```python
from build123d import *

# Parameters (mm, degrees)
SKETCH_1_W                    = 140
SKETCH_1_H                    = 140
EXTRUDE_1_DEPTH               = 24
SKETCH_2_R                    = 27.5
CUT_EXTRUDE_1_DEPTH           = 22
SKETCH_3_R                    = 24.5
CUT_EXTRUDE_2_DEPTH           = 102.410058673
HOLE_WIZARD_M10_1_D           = 12
HOLE_WIZARD_M10_1_CBORE_D     = 18
HOLE_WIZARD_M10_1_CBORE_DEPTH = 10.6
CHAMFER_1_SIZE                = 10
HOLE_WIZARD_M6_1_D            = 5
SKETCH_11_R                   = 40
CUT_EXTRUDE_3_DEPTH           = 9


with BuildPart() as part:
    # 草图1 → 凸台-拉伸1 (new body)
    with BuildSketch(Plane.XY):
        Rectangle(SKETCH_1_W, SKETCH_1_H)
    extrude(amount=EXTRUDE_1_DEPTH)

    # 草图2 → 切除-拉伸1 (cut)
    with BuildSketch(Plane(origin=(0, 0, 0), x_dir=(-1, 0, 0), z_dir=(0, 0, -1))):
        Circle(SKETCH_2_R)
    extrude(amount=-CUT_EXTRUDE_1_DEPTH, mode=Mode.SUBTRACT)

    # 草图3 → 切除-拉伸2 (cut, through all)
    with BuildSketch(Plane(origin=(0, 0, 22), x_dir=(-1, 0, 0), z_dir=(0, 0, -1))):
        Circle(SKETCH_3_R)
    extrude(amount=-CUT_EXTRUDE_2_DEPTH, mode=Mode.SUBTRACT)

    # M10 六角凹头螺钉的柱形沉头孔1 (through all)
    with Locations(Plane(origin=(0, 0, 0), x_dir=(-1, 0, 0), z_dir=(0, 0, -1))):
        with Locations((-52.5, 52.5), (52.5, 52.5), (52.5, -52.5), (-52.5, -52.5)):
            CounterBoreHole(HOLE_WIZARD_M10_1_D / 2, HOLE_WIZARD_M10_1_CBORE_D / 2, HOLE_WIZARD_M10_1_CBORE_DEPTH)

    # 倒角1
    chamfer_1_edges = [part.edges().sort_by_distance(p)[0] for p in [
        (70, -70, 12),
        (-70, -70, 12),
        (-70, 70, 12),
        (70, 70, 12),
    ]]
    chamfer(chamfer_1_edges, length=CHAMFER_1_SIZE)

    # M6 螺纹孔1 (through all)
    with Locations(Plane(origin=(0, 0, 0), x_dir=(-1, 0, 0), z_dir=(0, 0, -1))):
        with Locations((-35, 35), (35, 35), (35, -35), (-35, -35), (0, 0)):
            Hole(HOLE_WIZARD_M6_1_D / 2)

    # 草图11 → 切除-拉伸3 (cut)
    with BuildSketch(Plane(origin=(0, 0, 0), x_dir=(-1, 0, 0), z_dir=(0, 0, -1))):
        Circle(SKETCH_11_R)
    extrude(amount=-CUT_EXTRUDE_3_DEPTH, mode=Mode.SUBTRACT)


solid = part.part
```
Read the model definition and answer for the solid it produces. Units are mm, in the model's axes. A direction names the side the tool comes from. Give positions to 0.01 mm unless a question says otherwise; leave off trailing zeros. Order: outer loops, then holes, each group sorted by start corner. A loop starts at its lowest first (then second) coordinate and runs counter-clockwise, first axis right, second up.
(1) For a pull along X with two mould halves and no side action, classify faces 3 (the cylindrical face through (46.506, -52.236, 17.394)), 4 (the flat face through (65, 65, 12)), 5 (the cylindrical face through (-58.494, -52.236, 17.394)), 6 (the flat face through (-1, 70, 12)) as released by +X, released by -X, zero draft, split by the parting line, or undercut.
(2) Find section A-A (y = 0). Give the vertices of the cut face in (x, z).
(3) Given pin 1 (15.5 mm diameter, centred on x = 52.5, y = -52.5, fed in from -Z), flat-ended and moving along its own axis, determine where the tip first touches the part or whether it passes through.
(4) Find section D-D (z = 16). Give the number of separate pieces and of enclosed holes in the cut face, plus the area to 3 significant figures.
(5) Find section C-C (y = 52.5). Give the vertices of the cut face in (x, z), plus the area to 3 significant figures.
(6) For faces 1 (the cylindrical face through (59.133, 58.583, 5.226)), 2 (the cylindrical face through (-32.69, 34.04, 12.17)), determine the directions among +Z, -Z, +X, -X, +Y, -Y from which every point of the face is accessible in a straight line to the end or side of a thin tool.
(7) Straight lines are drawn through the part: L1, parallel to Y at x = 52.5, z = 17.5; L2, parallel to Y at x = 35, z = 17.5; L3, parallel to Y at x = -35, z = 8. For each, find the intervals that lie inside material, in ascending order.
Result sheet:
1. face 3: undercut
1. face 4: released by +X
1. face 5: undercut
1. face 6: zero draft
2. outline: (-70, 0) - (-40, 0) - (-40, 9) - (-27.5, 9) - (-27.5, 22) - (-24.5, 22) - (-24.5, 24) - (-70, 24) - close; (24.5, 22) - (27.5, 22) - (27.5, 9) - (40, 9) - (40, 0) - (70, 0) - (70, 24) - (24.5, 24) - close
3. pin 1: stops at z = 10.6
4. separate pieces: 1
4. enclosed holes: 9
4. area: 16,500 mm2
5. outline: (-70, 0) - (-61.5, 0) - (-61.5, 10.6) - (-58.5, 10.6) - (-58.5, 24) - (-70, 24) - close; (-46.5, 10.6) - (-43.5, 10.6) - (-43.5, 0) - (43.5, 0) - (43.5, 10.6) - (46.5, 10.6) - (46.5, 24) - (-46.5, 24) - close; (58.5, 10.6) - (61.5, 10.6) - (61.5, 0) - (70, 0) - (70, 24) - (58.5, 24) - close
5. area: 2,660 mm2
6. face 1: -Z
6. face 2: +Z, -Z
7. L1: y = -70 to -58.5, -46.5 to 46.5, 58.5 to 70
7. L2: y = -70 to -37.5, -32.5 to 32.5, 37.5 to 70
7. L3: y = -70 to -37.5, -32.5 to -19.36, 19.36 to 32.5, 37.5 to 70
